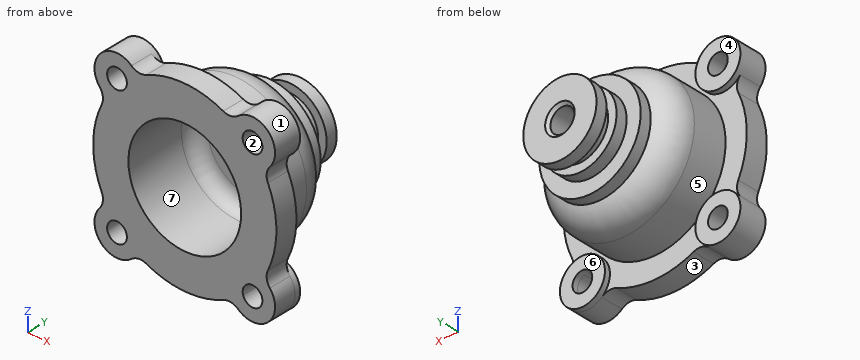
from build123d import *

# Parameters (mm, degrees)
M10_TAPPED_HOLE1_D  = 8.5
CHAMFER1_SIZE       = 1
SKETCH6_R           = 8
SKETCH6_R_2         = 3.5
BOSS_EXTRUDE1_DEPTH = 8
SKETCH7_R           = 3.5
CUT_EXTRUDE1_DEPTH  = 8
FILLET1_R           = 5
BOSS_EXTRUDE2_START = 2
SKETCH8_R           = 8
SKETCH8_R_2         = 3.5
BOSS_EXTRUDE2_DEPTH = 2


with BuildPart() as part:
    # Sketch1 → Revolve1 (revolve)
    with BuildSketch(Plane.XY, mode=Mode.PRIVATE) as revolve1_sk:
        with BuildLine():
            Line((0, 46), (-13, 46))
            Line((-13, 46), (-13, 42))
            Line((-13, 42), (-10, 42))
            Line((-10, 42), (-10, 38))
            Line((-10, 38), (-13, 38))
            Line((-13, 38), (-13, 34))
            Line((-13, 34), (-18, 34))
            Line((-18, 34), (-18, 30.006223624))
            ThreePointArc((-18, 30.006223624), (-23.062257748, 26.382911393), (-25, 20.46683161))
            Line((-25, 20.46683161), (-25, 8))
            Line((-25, 8), (-32.5, 8))
            Line((-32.5, 8), (-32.5, 0))
            Line((-32.5, 0), (-20, 0))
            Line((-20, 0), (-20, 21))
            ThreePointArc((-20, 21), (-18.535533906, 24.535533906), (-15, 26))
            Line((-15, 26), (0, 26))
            Line((0, 26), (0, 46))
        make_face()
    revolve(revolve1_sk.sketch.rotate(Axis((0, 0, 0), (0, 1, 0)), 270), axis=Axis((0, 0, 0), (0, 1, 0)))

    # M10 Tapped Hole1 (through all)
    with Locations(Plane(origin=(0, 46, 0), x_dir=(1, 0, 0), z_dir=(0, 1, 0))):
        with Locations((0, 0)):
            Hole(M10_TAPPED_HOLE1_D / 2)

    # Chamfer1
    chamfer1_edges = [part.edges().sort_by_distance(p)[0] for p in [
        (4.25, 46, 0),
    ]]
    chamfer(chamfer1_edges, length=CHAMFER1_SIZE)

    # Sketch6 → Boss-Extrude1 (add)
    # profile 1 of 4: a face of its own
    with BuildSketch(Plane(origin=(0, 8, 0), x_dir=(1, 0, 0), z_dir=(0, 1, 0))):
        with Locations((-24.04163056, 24.04163056)):
            Circle(SKETCH6_R)
        with Locations((-24.04163056, 24.04163056)):
            Circle(SKETCH6_R_2, mode=Mode.SUBTRACT)
    # profile 2 of 4: a face of its own
    with BuildSketch(Plane(origin=(0, 8, 0), x_dir=(1, 0, 0), z_dir=(0, 1, 0))):
        with Locations((24.04163056, 24.04163056)):
            Circle(SKETCH6_R)
        with Locations((24.04163056, 24.04163056)):
            Circle(SKETCH6_R_2, mode=Mode.SUBTRACT)
    # profile 3 of 4: a face of its own
    with BuildSketch(Plane(origin=(0, 8, 0), x_dir=(1, 0, 0), z_dir=(0, 1, 0))):
        with Locations((24.04163056, -24.04163056)):
            Circle(SKETCH6_R)
        with Locations((24.04163056, -24.04163056)):
            Circle(SKETCH6_R_2, mode=Mode.SUBTRACT)
    # profile 4 of 4: a face of its own
    with BuildSketch(Plane(origin=(0, 8, 0), x_dir=(1, 0, 0), z_dir=(0, 1, 0))):
        with Locations((-24.04163056, -24.04163056)):
            Circle(SKETCH6_R)
        with Locations((-24.04163056, -24.04163056)):
            Circle(SKETCH6_R_2, mode=Mode.SUBTRACT)
    extrude(amount=-BOSS_EXTRUDE1_DEPTH)

    # Sketch7 → Cut-Extrude1 (cut)
    with BuildSketch(Plane(origin=(0, 8, 0), x_dir=(1, 0, 0), z_dir=(0, 1, 0))):
        with Locations(Location((-24.04163056, 24.04163056, 0), (0, 0, 270))):
            Circle(SKETCH7_R)
        with Locations(Location((24.04163056, 24.04163056, 0), (0, 0, 270))):
            Circle(SKETCH7_R)
        with Locations(Location((24.04163056, -24.04163056, 0), (0, 0, 270))):
            Circle(SKETCH7_R)
        with Locations(Location((-24.04163056, -24.04163056, 0), (0, 0, 270))):
            Circle(SKETCH7_R)
    extrude(amount=-CUT_EXTRUDE1_DEPTH, mode=Mode.SUBTRACT)

    # Fillet1
    fillet1_edges = [part.edges().sort_by_distance(p)[0] for p in [
        (-16.944361965, 4, -27.733348113),
        (-27.733348113, 4, -16.944361965),
        (-27.733348113, 4, 16.944361965),
        (-16.944361965, 4, 27.733348113),
        (16.944361965, 4, 27.733348113),
        (27.733348113, 4, 16.944361965),
        (27.733348113, 4, -16.944361965),
        (16.944361965, 4, -27.733348113),
    ]]
    fillet(fillet1_edges, radius=FILLET1_R)

    # Sketch8 → Boss-Extrude2 (add)
    # profile 1 of 4: a face of its own
    with BuildSketch(Plane(origin=(0, 8, 0), x_dir=(1, 0, 0), z_dir=(0, 1, 0)).offset(BOSS_EXTRUDE2_START)):
        with Locations(Location((-24.04163056, 24.04163056, 0), (0, 0, 270))):
            Circle(SKETCH8_R)
        with Locations(Location((-24.04163056, 24.04163056, 0), (0, 0, 270))):
            Circle(SKETCH8_R_2, mode=Mode.SUBTRACT)
    # profile 2 of 4: a face of its own
    with BuildSketch(Plane(origin=(0, 8, 0), x_dir=(1, 0, 0), z_dir=(0, 1, 0)).offset(BOSS_EXTRUDE2_START)):
        with Locations(Location((24.04163056, 24.04163056, 0), (0, 0, 270))):
            Circle(SKETCH8_R)
        with Locations(Location((24.04163056, 24.04163056, 0), (0, 0, 270))):
            Circle(SKETCH8_R_2, mode=Mode.SUBTRACT)
    # profile 3 of 4: a face of its own
    with BuildSketch(Plane(origin=(0, 8, 0), x_dir=(1, 0, 0), z_dir=(0, 1, 0)).offset(BOSS_EXTRUDE2_START)):
        with Locations(Location((24.04163056, -24.04163056, 0), (0, 0, 270))):
            Circle(SKETCH8_R)
        with Locations(Location((24.04163056, -24.04163056, 0), (0, 0, 270))):
            Circle(SKETCH8_R_2, mode=Mode.SUBTRACT)
    # profile 4 of 4: a face of its own
    with BuildSketch(Plane(origin=(0, 8, 0), x_dir=(1, 0, 0), z_dir=(0, 1, 0)).offset(BOSS_EXTRUDE2_START)):
        with Locations(Location((-24.04163056, -24.04163056, 0), (0, 0, 270))):
            Circle(SKETCH8_R)
        with Locations(Location((-24.04163056, -24.04163056, 0), (0, 0, 270))):
            Circle(SKETCH8_R_2, mode=Mode.SUBTRACT)
    extrude(amount=-BOSS_EXTRUDE2_DEPTH)


solid = part.part
The model under review builds one solid part; all positions refer to its coordinate system, in mm. Face numbers are marked on the shaded views. A direction names the side the tool comes from. Round coordinates to 2 decimals unless told otherwise and drop trailing zeros. Loops run counter-clockwise (first coordinate to the right, second up) from the corner with the lowest first, then second, coordinate; pieces in that order, holes last. Notation, with made-up numbers: M -1,31.25 L 46,31.25 A19 cw 46,59.25 Z; hole C -30.75,54.25 d5. An arc over 180 degrees is marked long. Answer as CSV lines item,"result". Start each with the question number.
Item 1: Insertion check: P1, Ø5, axis at x = 27, z = -22, coming from the +Y side; P2, Ø12, axis at y = 29.5, z = -23, coming from the +X side; P3, Ø2, axis at x = 13, y = 30, coming from the -Z side. Each pin has a flat end and moves straight along its axis. Give the tip position at first contact, or say it passes through.
Item 2: Consider section B-B (y = 37). Write out the cut boundary in (x, z).
Item 3: Consider section A-A (y = 15). Write out the cut boundary in (x, z).
Item 4: Mouldability with a two-part tool opening along Z and no side actions: class the marked faces 1, 2, 3 and 4 as released by +Z, released by -Z, zero draft, split by the parting line, or undercut.
Item 5: Consider section C-C (y = 6.5). State how many separate pieces and enclosed holes the cut face has, then the cut area to 3 significant figures.
Item 6: For the marked faces 5, 6 and 7, list the 3-axis set-ups (+Z, -Z, +X, -X, +Y, -Y) from which the entire face can be reached by the end or side of a thin tool; tool diameter is ignored.
Item 7: Wall thickness on line 1 (Y direction, x = -21, z = -17); line 2 (Y direction, x = 6.5, z = 1); line 3 (X direction, y = 9, z = 0): over which ranges is each line inside the solid? List them lowest first. Write a range as [from, to].
Answer:
1,P1,"stops at y = 10"
1,P2,"stops at x = 14.71"
1,P3,"stops at z = -15.63"
2,outline,"C 0,0 d26; hole C 0,0 d8.5"
3,outline,"C 0,0 d50; hole C 0,0 d40"
4,face 1,"undercut"
4,face 2,"undercut"
4,face 3,"released by -Z"
4,face 4,"zero draft"
5,separate pieces,"1"
5,enclosed holes,"5"
5,area,"2,450 mm^2"
6,face 5,"+Y"
6,face 6,"-Z, +X, +Y"
6,face 7,"-Y"
7,line 1,"y = [0, 10]"
7,line 2,"y = [26, 46]"
7,line 3,"x = [-25, -20], [20, 25]"
